from build123d import *

# Parameters (mm, degrees)
SKETCH2_R           = 14.1
BOSS_EXTRUDE2_DEPTH = 14


with BuildPart() as part:
    # Sketch2 → Boss-Extrude2 (new body)
    with BuildSketch(Plane.XY):
        with BuildLine():
            Line((10, 181), (10, 196))
            ThreePointArc((10, 196), (11.464466094, 199.535533906), (15, 201))
            Line((15, 201), (25.209501406, 201))
            ThreePointArc((25.209501406, 201), (33.408153022, 198.561134968), (38.940750673, 192.037614891))
            Line((38.940750673, 192.037614891), (76.997541741, 40))
            Line((76.997541741, 40), (76.997541741, 30))
            Line((76.997541741, 30), (76.997541741, 10))
            Line((76.997541741, 10), (76.997541741, 0))
            Line((76.997541741, 0), (20, 0))
            ThreePointArc((20, 0), (12.928932188, 2.928932188), (10, 10))
            Line((10, 10), (10, 21))
            Line((10, 21), (0, 21))
            Line((0, 21), (0, 41))
            Line((0, 41), (10, 41))
            Line((10, 41), (10, 101))
            Line((10, 101), (10, 161))
            Line((10, 161), (0, 161))
            Line((0, 161), (0, 181))
            Line((0, 181), (10, 181))
        make_face()
        with Locations((48, 21)):
            Circle(SKETCH2_R, mode=Mode.SUBTRACT)
    extrude(amount=BOSS_EXTRUDE2_DEPTH)


solid = part.part
Design review of the part built by this model. Coordinates are the model's own, in mm. A direction names the side the tool comes from. Coordinates: 2 decimals unless noted, no trailing zeros. Write each loop counter-clockwise with the first axis right and the second up, starting at its lowest first coordinate (ties: lowest second). Pieces come first, ordered by that corner, then holes. Notation, with made-up numbers: (85.5, -33) - (111.5, -33) arc R30 cw to (111.5, -11) - close; hole circle Ø3 at (33.5, -27.5). An arc over 180 degrees is marked (long way). Use one line per item in the form item = value.
Q1. Consider section C-C (z = 10.25). Write out the cut boundary in (x, y).
Taken from the geometry:
outline = (0, 21) - (10, 21) - (10, 10) arc R10 ccw to (20, 0) - (77, 0) - (77, 40) - (38.94, 192.04) arc R15 ccw to (25.21, 201) - (15, 201) arc R5 ccw to (10, 196) - (10, 181) - (0, 181) - (0, 161) - (10, 161) - (10, 41) - (0, 41) - close; hole circle Ø28.2 at (48, 21)
Q2. Machinability: for faces 5 (the flat face through (10, 188, 7)), 6 (the flat face through (10, 15, 7)), 7 (the flat face through (5, 41, 7)), which of the approach directions +Z, -Z, +X, -X, +Y, -Y give a long, thin tool a straight path to every point of the face, cutting with its end or side? Answer none if there is none.
Taken from the geometry:
face_5 = +Z, -Z, -X, +Y
face_6 = +Z, -Z, -X, -Y
face_7 = +Z, -Z, -X
Q3. The part is to be moulded in two halves that separate along Y. For faces 1 (the flat face through (5, 161, 7)), 2 (the flat face through (57.7, 117.1, 6.9)), 3 (the flat face through (5, 21, 7)), 4 (the cylindrical face through (36.81, 12.42, 6.9)), say which applies: +Y half, -Y half, draft (parallel to the pull), parting line (faces both ways), or undercut.
Taken from the geometry:
face_1 = undercut
face_2 = +Y half
face_3 = -Y half
face_4 = undercut
Q4. Insertion check: pin 1 Ø5 at (x, z) = (7, 7) entering from -Y; pin 2 Ø3.5 at (y, z) = (16.5, 8) entering from -X; pin 3 Ø6 at (x, y) = (62, 21) entering from -Z; pin 4 Ø3 at (x, z) = (2.5, 4.5) entering from +Y. Each pin has a flat end and moves straight along its axis. Give the tip position at first contact, or say it passes through.
Taken from the geometry:
pin_1 = 21
pin_2 = 10
pin_3 = 0
pin_4 = 181
Q5. Consider section A-A (x = 6). Write out the cut boundary in (y, z).
Taken from the geometry:
outline = (21, 0) - (41, 0) - (41, 14) - (21, 14) - close; (161, 0) - (181, 0) - (181, 14) - (161, 14) - close
Q6. Consider section B-B (y = 30). Write out the cut boundary in (x, z), plus the area to 3 significant figures.
Taken from the geometry:
outline = (0, 0) - (37.15, 0) - (37.15, 14) - (0, 14) - close; (58.85, 0) - (77, 0) - (77, 14) - (58.85, 14) - close
area = 774 mm^2
Q7. Consider section D-D (y = 103.5). Write out the cut boundary in (x, z), plus the area to 3 significant figures.
Taken from the geometry:
outline = (10, 0) - (61.1, 0) - (61.1, 14) - (10, 14) - close
area = 715 mm^2
Q8. For probe 1 along X at (y, z) = (14.5, 7); probe 2 along X at (y, z) = (8, 12.5); probe 3 along Y at (x, z) = (15, 12.25), list the stretches that pass through material, from the lowest coordinate up.
Taken from the geometry:
probe_1 = 10 to 35.49, 60.51 to 77
probe_2 = 10.2 to 42.54, 53.46 to 77
probe_3 = 1.34 to 201
